Study the drawing (mm; zero at the part's minimum x, y, z) and answer. Give positions to 0.01 mm unless a question says otherwise; leave off trailing zeros. Loops run counter-clockwise (first coordinate to the right, second up) from the corner with the lowest first, then second, coordinate; pieces in that order, holes last. Notation, with made-up numbers: (-24, 21.25) - (-18, 21.25) arc R24 ccw to (-18, 40.25) - close; hole circle Ø9 at (41.25, -31). An arc over 180 degrees is marked (long way). Answer in a Markdown table with one row per item. Add a question column.
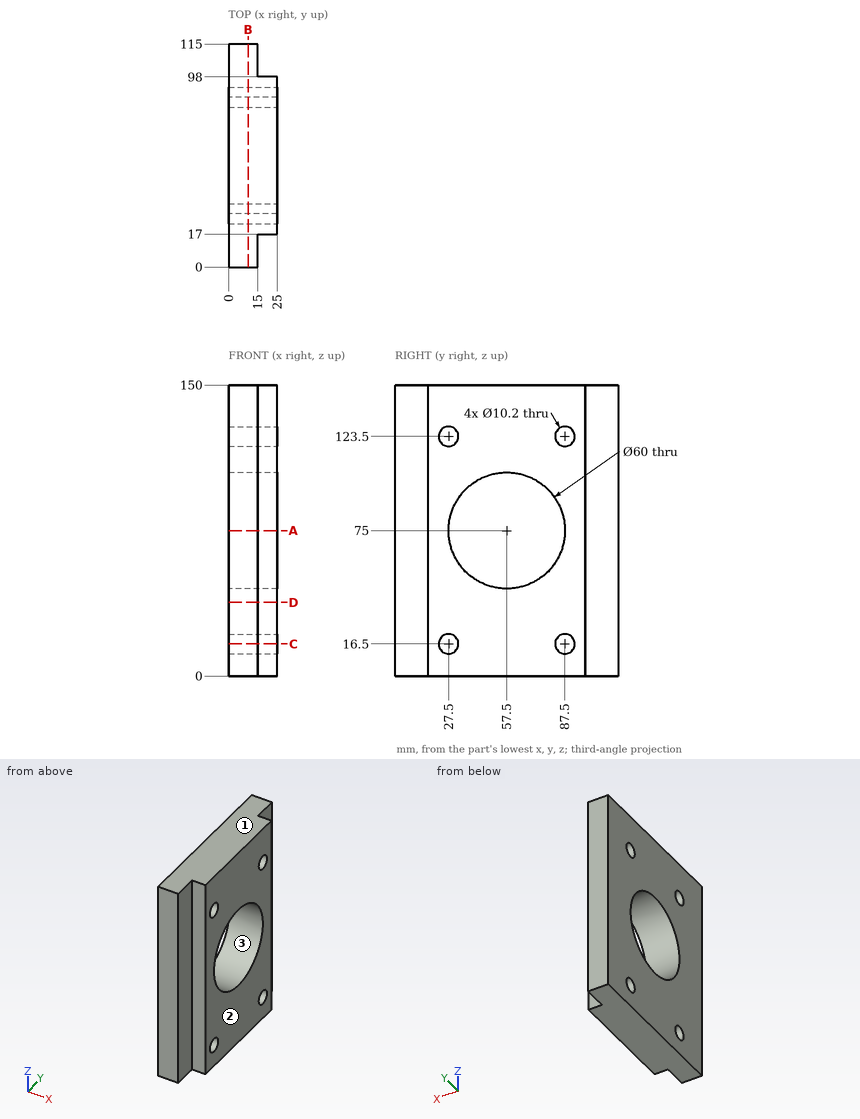
(1) The mould has two halves that part along Z. Classify the marked faces 1, 2 and 3: pulls with the +Z half, pulls with the -Z half, needs draft (parallel to the pull), parting line crosses it, or undercut.
(2) Given pin 1 Ø9 at (y, z) = (87.5, 123.5) entering from +X; pin 2 Ø13.5 at (y, z) = (5.5, 93.5) entering from +X; pin 3 Ø11 at (x, z) = (22, 46.5) entering from -Y, each flat-ended and moving along its own axis, determine where each tip first touches the part or whether it passes through.
(3) Find the intervals of material crossed by line 1 along Y through (x, z) = (13.5, 16.5); line 2 along Y through (x, z) = (16.75, 123.5); line 3 along Z through (x, y) = (15.75, 91.5), in increasing order. Write a range as [from, to].
(4) A cutting plane is placed at B-B on x = 10. Determine the outline of the cut face in (y, z).
(5) A cutting plane is placed at C-C on z = 16.5. Determine the outline of the cut face in (x, y).
(6) A cutting plane is placed at D-D on z = 38. Determine the outline of the cut face in (x, y), plus the area to 4 significant figures.
(7) A cutting plane is placed at A-A on z = 75. Determine the outline of the cut face in (x, y), plus the area to 4 significant figures.
Evaluation:
| question | item | result |
|---|---|---|
| 1 | face 1 | pulls with the +Z half |
| 1 | face 2 | needs draft |
| 1 | face 3 | undercut |
| 2 | pin 1 | passes through |
| 2 | pin 2 | stops at x = 15 |
| 2 | pin 3 | stops at y = 17 |
| 3 | line 1 | y = [0, 22.4], [32.6, 82.4], [92.6, 115] |
| 3 | line 2 | y = [17, 22.4], [32.6, 82.4], [92.6, 98] |
| 3 | line 3 | z = [0, 13.34], [19.66, 120.34], [126.66, 150] |
| 4 | outline | (0, 0) - (115, 0) - (115, 150) - (0, 150) - close; hole circle Ø10.2 at (27.5, 16.5); hole circle Ø10.2 at (27.5, 123.5); hole circle Ø60 at (57.5, 75); hole circle Ø10.2 at (87.5, 16.5); hole circle Ø10.2 at (87.5, 123.5) |
| 5 | outline | (0, 0) - (15, 0) - (15, 17) - (25, 17) - (25, 22.4) - (0, 22.4) - close; (0, 32.6) - (25, 32.6) - (25, 82.4) - (0, 82.4) - close; (0, 92.6) - (25, 92.6) - (25, 98) - (15, 98) - (15, 115) - (0, 115) - close |
| 6 | outline | (0, 0) - (15, 0) - (15, 17) - (25, 17) - (25, 98) - (15, 98) - (15, 115) - (0, 115) - close |
| 6 | area | 2,535 mm² |
| 7 | outline | (0, 0) - (15, 0) - (15, 17) - (25, 17) - (25, 27.5) - (0, 27.5) - close; (0, 87.5) - (25, 87.5) - (25, 98) - (15, 98) - (15, 115) - (0, 115) - close |
| 7 | area | 1,035 mm² |
